Study the drawing (mm; zero at the part's minimum x, y, z) and answer. Round coordinates to 2 decimals unless told otherwise and drop trailing zeros. Loops run counter-clockwise (first coordinate to the right, second up) from the corner with the lowest first, then second, coordinate; pieces in that order, holes last. Notation, with made-up numbers: (14.5, -26.75) - (30.5, -26.75) arc R25 cw to (30.5, 1.25) - close; hole circle Ø10 at (12.25, -5.5). An arc over 180 degrees is marked (long way). Use CSV: the item, a comma, the result in double quotes. Start each with the question number.
1. Determine the mould class of the marked faces 1, 2 and 3 for opening direction Y: +Y half, -Y half, draft (parallel to the pull), parting line (faces both ways), or undercut.
2. Consider line 1 along Y through (x, z) = (60, 39); line 2 along Z through (x, y) = (7, 39.5); line 3 along X through (y, z) = (43, 97). Determine where each line is inside the solid, lowest interval first.
3. Given pin 1 Ø3 at (y, z) = (25, 25) entering from -X; pin 2 Ø6 at (x, z) = (85.5, 84.5) entering from -Y; pin 3 Ø1.5 at (x, z) = (16.5, 69.5) entering from -Y, each flat-ended and moving along its own axis, determine where each tip first touches the part or whether it passes through.
4. Find section C-C (z = 48). Give the vertices of the cut face in (x, y).
5. Find section A-A (x = 60). Give the vertices of the cut face in (y, z).
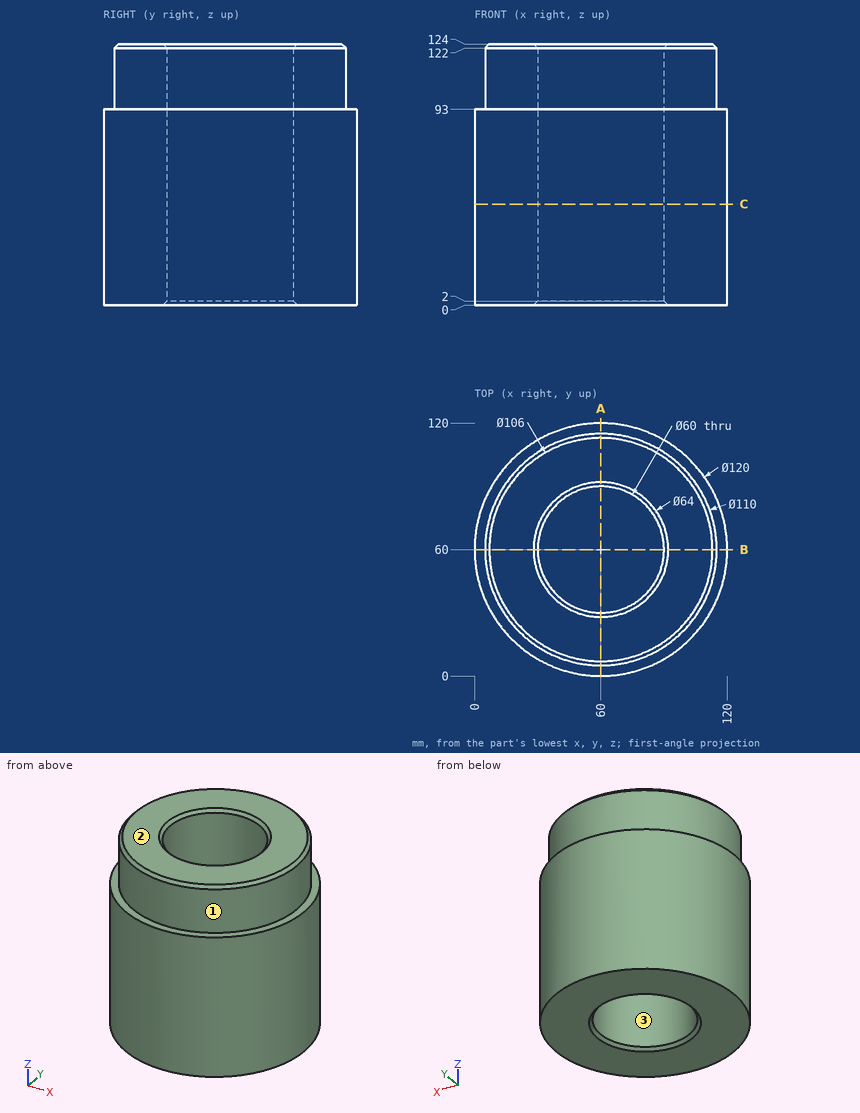
Filled sheet:
1,face 1,"parting line"
1,face 2,"draft"
1,face 3,"undercut"
2,line 1,"y = 0 to 30, 90 to 120"
2,line 2,"z = 0 to 93"
2,line 3,"x = 7.69 to 35.28, 84.72 to 112.31"
3,pin 1,"stops at x = 10.22"
3,pin 2,"stops at y = 4.38"
3,pin 3,"stops at y = 17.9"
4,outline,"circle Ø120 at (60, 60); hole circle Ø60 at (60, 60)"
5,outline,"(0, 0) - (28, 0) - (30, 2) - (30, 122) - (28, 124) - (7, 124) - (5, 122) - (5, 93) - (0, 93) - close; (90, 2) - (92, 0) - (120, 0) - (120, 93) - (115, 93) - (115, 122) - (113, 124) - (92, 124) - (90, 122) - close"
